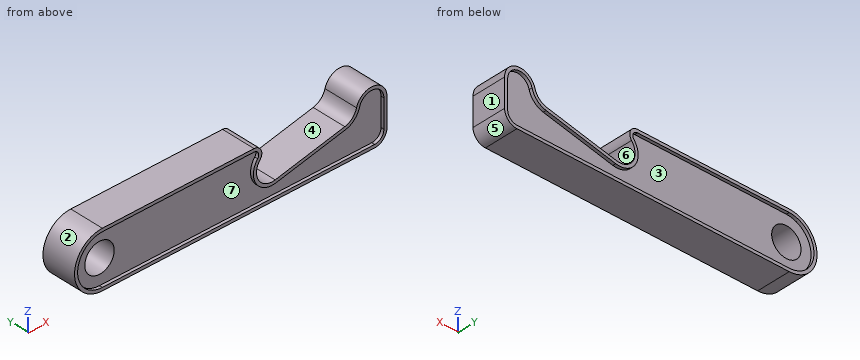
```python
from build123d import *

# Parameters (mm, degrees)
LEVER_PROFILE_SKETCH_R    = 4.75
LEVER_BODY_11MM_DEPTH     = 5.5
TOP_FACE_RECESS_1MM_DEPTH = 1


with BuildPart() as part:
    # Lever Profile Sketch → Lever Body 11mm (new, symmetric)
    with BuildSketch(Plane(origin=(0, 0, 0), x_dir=(1, 0, 0), z_dir=(0, 1, 0))):
        with BuildLine():
            Line((46.5, 9), (-41.5, 9))
            ThreePointArc((-41.5, 9), (-50.5, 0), (-41.5, -9))
            Line((-41.5, -9), (7.540217235, -9))
            ThreePointArc((7.540217235, -9), (9.802454571, -7.564087513), (9.465992035, -4.905825787))
            ThreePointArc((9.465992035, -4.905825787), (9.040307373, 0.871975682), (14.357100089, 3.173260641))
            Line((14.357100089, 3.173260641), (36.857100089, -1.609261996))
            ThreePointArc((36.857100089, -1.609261996), (39.275815642, -2.888858783), (40.658770817, -5.25))
            ThreePointArc((40.658770817, -5.25), (46.130021462, -8.960148481), (50.5, -4))
            Line((50.5, -4), (50.5, 5))
            ThreePointArc((50.5, 5), (49.328427125, 7.828427125), (46.5, 9))
        make_face()
        with Locations(Location((-41.5, 0, 0), (0, 0, 270))):
            Circle(LEVER_PROFILE_SKETCH_R, mode=Mode.SUBTRACT)
    extrude(amount=LEVER_BODY_11MM_DEPTH, both=True)

    # Face Recess Sketch → Top Face Recess 1mm (cut)
    with BuildSketch(Plane(origin=(0, 5.5, 0), x_dir=(1, 0, 0), z_dir=(0, 1, 0))):
        with BuildLine():
            Line((-41.5, -8), (7.540217235, -8))
            ThreePointArc((7.540217235, -8), (8.897559636, -7.138452508), (8.695682115, -5.543495472))
            ThreePointArc((8.695682115, -5.543495472), (8.18486052, 1.389866291), (14.565011779, 4.151408242))
            Line((14.565011779, 4.151408242), (37.065011779, -0.631114396))
            ThreePointArc((37.065011779, -0.631114396), (39.967470443, -2.166630539), (41.627016654, -5))
            ThreePointArc((41.627016654, -5), (46.00401717, -7.968118785), (49.5, -4))
            Line((49.5, -4), (49.5, 5))
            ThreePointArc((49.5, 5), (48.621320344, 7.121320344), (46.5, 8))
            Line((46.5, 8), (-41.5, 8))
            ThreePointArc((-41.5, 8), (-49.5, 0), (-41.5, -8))
        make_face()
    top_face_recess_1mm = extrude(amount=-TOP_FACE_RECESS_1MM_DEPTH, mode=Mode.SUBTRACT)

    # Bottom Face Recess Mirror: Top Face Recess 1mm across plane
    add(top_face_recess_1mm.mirror(Plane.ZX), mode=Mode.SUBTRACT)


solid = part.part
```
Read the model definition and answer for the solid it produces. Units are mm, in the model's axes. Face numbers are marked on the shaded views. A direction names the side the tool comes from. Give positions to 0.01 mm unless a question says otherwise; leave off trailing zeros. Order: outer loops, then holes, each group sorted by start corner. A loop starts at its lowest first (then second) coordinate and runs counter-clockwise, first axis right, second up.
(1) For the marked faces 4, 5, 6 and 7, determine the directions among +Z, -Z, +X, -X, +Y, -Y from which every point of the face is accessible in a straight line to the end or side of a thin tool.
(2) Find section C-C (x = -15.5). Give the vertices of the cut face in (y, z), plus the area to 3 significant figures.
(3) Find section A-A (z = 2.5). Give the vertices of the cut face in (x, y).
(4) For a pull along X with two mould halves and no side action, classify the marked faces 1, 2 and 3 as released by +X, released by -X, zero draft, split by the parting line, or undercut.
(5) Find section B-B (y = -2.25). Give the vertices of the cut face in (x, z), plus the area to 3 significant figures.
(6) Find section D-D (z = -6). Give the vertices of the cut face in (x, y), plus the area to 3 significant figures.
(7) Straight lines are drawn through the part: L1, parallel to Z at x = -41.5, y = -2; L2, parallel to X at y = 3, z = 2; L3, parallel to X at y = -3.5, z = 3.75. For each, find the intervals that lie inside material, in ascending order.
(8) Given pin 1 (8 mm diameter, centred on x = -3, z = -2, fed in from -Y); pin 2 (1 mm diameter, centred on y = -2, z = -5, fed in from -X); pin 3 (1.1 mm diameter, centred on y = -5, z = 1.5, fed in from -X); pin 4 (5 mm diameter, centred on x = 29.5, z = 2, fed in from +Y), each flat-ended and moving along its own axis, determine where each tip first touches the part or whether it passes through.
Result sheet:
1. face 4: +Z, +Y, -Y
1. face 5: -Z, +X, +Y, -Y
1. face 6: +Y, -Y
1. face 7: -Y
2. outline: (-5.5, -9) - (5.5, -9) - (5.5, -8) - (4.5, -8) - (4.5, 8) - (5.5, 8) - (5.5, 9) - (-5.5, 9) - (-5.5, 8) - (-4.5, 8) - (-4.5, -8) - (-5.5, -8) - close
2. area: 166 mm2
3. outline: (-50.15, -5.5) - (-49.1, -5.5) - (-49.1, -4.5) - (-45.54, -4.5) - (-45.54, 4.5) - (-49.1, 4.5) - (-49.1, 5.5) - (-50.15, 5.5) - close; (-37.46, -4.5) - (7.37, -4.5) - (7.37, -5.5) - (8.38, -5.5) - (8.38, 5.5) - (7.37, 5.5) - (7.37, 4.5) - (-37.46, 4.5) - close; (38.82, -5.5) - (40.29, -5.5) - (40.29, -4.5) - (49.5, -4.5) - (49.5, -5.5) - (50.5, -5.5) - (50.5, 5.5) - (49.5, 5.5) - (49.5, 4.5) - (40.29, 4.5) - (40.29, 5.5) - (38.82, 5.5) - close
4. face 1: released by +X
4. face 2: released by -X
4. face 3: undercut
5. outline: (-41.5, -9) - (46.5, -9) arc R4 ccw to (50.5, -5) - (50.5, 4) arc R5 ccw to (40.66, 5.25) arc R5 cw to (36.86, 1.61) - (14.36, -3.17) arc R5 cw to (9.47, 4.91) arc R2.5 ccw to (7.54, 9) - (-41.5, 9) arc R9 ccw to start; hole circle Ø9.5 at (-41.5, 0)
5. area: 1,390 mm2
6. outline: (-48.21, -5.5) - (-46.79, -5.5) - (-46.79, -4.5) - (49.33, -4.5) - (49.33, -5.5) - (50.37, -5.5) - (50.37, 5.5) - (49.33, 5.5) - (49.33, 4.5) - (-46.79, 4.5) - (-46.79, 5.5) - (-48.21, 5.5) - close
6. area: 892 mm2
7. L1: z = -9 to -4.75, 4.75 to 9
7. L2: x = -50.27 to -45.81, -37.19 to 8.33, 38 to 50.5
7. L3: x = -49.68 to -44.42, -38.58 to 8.75, 39.99 to 50.5
8. pin 1: stops at y = -4.5
8. pin 2: stops at x = -49.29
8. pin 3: stops at x = -50.45
8. pin 4: stops at y = 5.5
